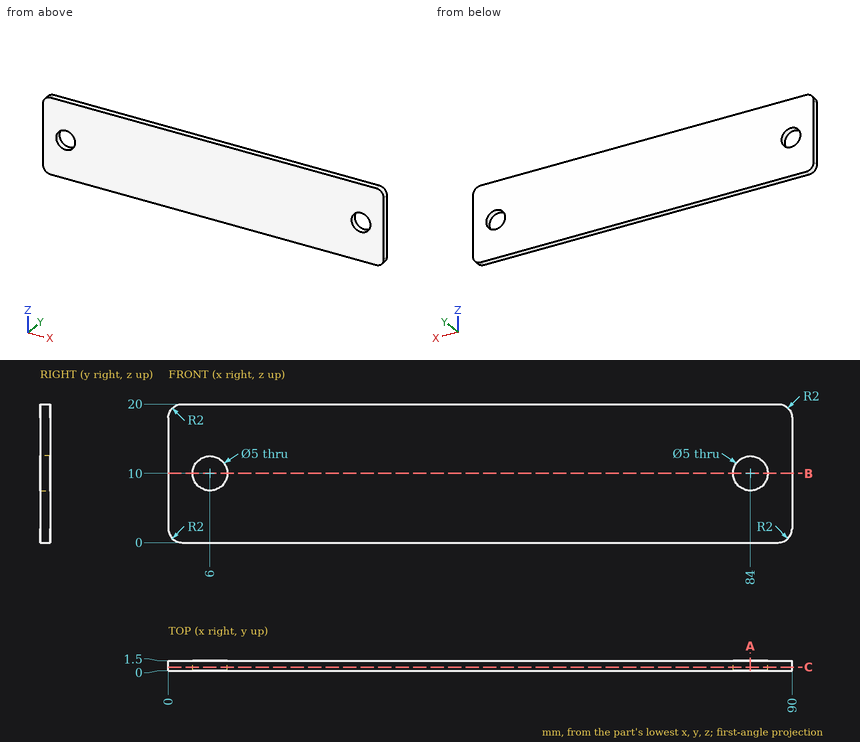
Drawing for the job (mm, zero at the part's lowest x, y, z). Give positions to 0.01 mm unless a question says otherwise; leave off trailing zeros. Loops run counter-clockwise (first coordinate to the right, second up) from the corner with the lowest first, then second, coordinate; pieces in that order, holes last.
Item 1: Slice it at C-C (y = 0.55). Write the cut outline in (x, z), plus the area to 3 significant figures.
Check values:
outline: (0, 2) arc R2 ccw to (2, 0) - (88, 0) arc R2 ccw to (90, 2) - (90, 18) arc R2 ccw to (88, 20) - (2, 20) arc R2 ccw to (0, 18) - close; hole circle Ø5 at (6, 10); hole circle Ø5 at (84, 10)
area: 1,760 mm2
Item 2: Drill centre lines: line 1 along X through (y, z) = (1.1, 10); line 2 along X through (y, z) = (0.75, 10.5); line 3 along Z through (x, y) = (82, 0.4). Where is each one in solid material? Low to high.
Check values:
line 1: x = 0 to 3.5, 8.5 to 81.5, 86.5 to 90
line 2: x = 0 to 3.55, 8.45 to 81.55, 86.45 to 90
line 3: z = 0 to 8.5, 11.5 to 20
Item 3: Slice it at A-A (x = 84). Write the cut outline in (y, z).
Check values:
outline: (0, 0) - (1.5, 0) - (1.5, 7.5) - (0, 7.5) - close; (0, 12.5) - (1.5, 12.5) - (1.5, 20) - (0, 20) - close
Item 4: Slice it at B-B (z = 10). Write the cut outline in (x, y), plus the area to 3 significant figures.
Check values:
outline: (0, 0) - (3.5, 0) - (3.5, 1.5) - (0, 1.5) - close; (8.5, 0) - (81.5, 0) - (81.5, 1.5) - (8.5, 1.5) - close; (86.5, 0) - (90, 0) - (90, 1.5) - (86.5, 1.5) - close
area: 120 mm2
